Design review of the part built by this model. Coordinates are the model's own, in mm. A direction names the side the tool comes from. Coordinates: 2 decimals unless noted, no trailing zeros. Write each loop counter-clockwise with the first axis right and the second up, starting at its lowest first coordinate (ties: lowest second). Pieces come first, ordered by that corner, then holes.
Q1. The part is to be moulded in two halves that separate along Y. For faces 4 (the face through (1.126, -18.148, 7.591)), 5 (the face through (-24, -124, 40.25)), 6 (the face through (-24.77, -126.96, 24.55)), say which applies: +Y half, -Y half, draft (parallel to the pull), parting line (faces both ways), or undercut.
Q2. Machinability: for faces 1 (the face through (1.293, -5.751, 6.201)), 2 (the face through (-24.2, -127.2, 10.25)), 3 (the face through (-7.065, -77.672, 9.667)), which of the approach directions +Z, -Z, +X, -X, +Y, -Y give a long, thin tool a straight path to every point of the face, cutting with its end or side? Answer none if there is none.
Q3. To check wall thickness, follow probe 1 along Y at (x, z) = (-24, 15.5); probe 2 along Z at (x, y) = (-5.5, -71); probe 3 along Y at (x, z) = (-23, 32). State the ranges of each line that lie inside material, in increasing order.
Q4. Add section B-B, the plane z = 34. Give the boundary of the cut face in (x, y), plus the area to 3 significant figures.
Q5. Clearance check with flat-ended pins moving along their axes: pin 1 Ø4 at (x, z) = (-22.5, 29) entering from -Y; pin 2 Ø8 at (x, y) = (-9.5, -81.5) entering from +Z; pin 3 Ø8 at (x, y) = (-25, -122.5) entering from -Z. State where each tip first meets the part, or that it passes through.
Q6. Add section A-A, the plane y = 0. Give the boundary of the cut face in (x, z).
from build123d import *

# Parameters (mm, degrees)
SKETCH1_R           = 9.25
SKETCH1_R_2         = 6.25
BOSS_EXTRUDE1_DEPTH = 12.5
SWEEP1_PROFILE_R    = 3.5
SKETCH16_R          = 5
BOSS_EXTRUDE2_DEPTH = 4
SKETCH17_R          = 3.096104317
BOSS_EXTRUDE3_DEPTH = 30
CHAMFER1_SIZE       = 1


with BuildPart() as part:
    # Sketch1 → Boss-Extrude1 (new body)
    with BuildSketch(Plane.XY):
        Circle(SKETCH1_R)
        Circle(SKETCH1_R_2, mode=Mode.SUBTRACT)
    extrude(amount=BOSS_EXTRUDE1_DEPTH)

    # Sweep1: sweep along a curve in space
    with BuildLine() as sweep1_path:
        Line((0, -6.25, 6.25), (7.675401854, -26.137831295, 6.25))
        ThreePointArc((7.782428128, -33.048212427, 6.25), (8.344876366, -29.583482004, 6.25), (7.675401854, -26.137831295, 6.25))
        Line((7.782428128, -33.048212427, 6.25), (-24.097440523, -123.936842128, 6.25))
    # Sweep1 profile (on start of the path) → Sweep1 (sweep)
    with BuildSketch(Plane(origin=(0, -6.25, 6.25), x_dir=(-0.9329326350915154, -0.36005096636615397, 0), z_dir=(0.36005096636615397, -0.9329326350915154, 0))):
        Circle(SWEEP1_PROFILE_R)
    sweep(path=sweep1_path.line)

    # Sketch16 → Boss-Extrude2 (add, symmetric)
    with BuildSketch(Plane.XY.offset(6.25)):
        with Locations((-24.097440523, -123.936842128)):
            Circle(SKETCH16_R)
    extrude(amount=BOSS_EXTRUDE2_DEPTH, both=True)

    # Sketch17 → Boss-Extrude3 (add)
    with BuildSketch(Plane.XY.offset(10.25)):
        with Locations((-24.097440523, -123.936842128)):
            Circle(SKETCH17_R)
    extrude(amount=BOSS_EXTRUDE3_DEPTH)

    # Chamfer1
    chamfer1_edges = [part.edges().sort_by_distance(p)[0] for p in [
        (-27.19354484, -123.936842128, 40.25),
    ]]
    chamfer(chamfer1_edges, length=CHAMFER1_SIZE)


solid = part.part
Here are the results:
1. face 4: undercut
1. face 5: draft
1. face 6: parting line
2. face 1: +Z, -Z
2. face 2: +Z
2. face 3: none
3. probe 1: y = -127.03 to -120.84
3. probe 2: z = 2.75 to 9.75
3. probe 3: y = -126.83 to -121.04
4. outline: circle Ø6.19 at (-24.1, -123.94)
4. area: 30.1 mm2
5. pin 1: stops at y = -127.03
5. pin 2: stops at z = 9.75
5. pin 3: stops at z = 2.25
6. outline: (-9.25, 0) - (-6.25, 0) - (-6.25, 12.5) - (-9.25, 12.5) - close; (6.25, 0) - (9.25, 0) - (9.25, 12.5) - (6.25, 12.5) - close
